Input: dimensioned drawing with shaded views. Units: mm. Origin: part minimum x, y, z. A direction names the side the tool comes from. Round coordinates to 2 decimals unless told otherwise and drop trailing zeros. Loops run counter-clockwise (first coordinate to the right, second up) from the corner with the lowest first, then second, coordinate; pieces in that order, holes last. Notation, with made-up numbers: (-3, 60.25) - (5, 60.25) arc R21 ccw to (5, 68.25) - close; hole circle Ø3 at (25.5, 39.25). An arc over 180 degrees is marked (long way). One line per question, with ' | ' between items.
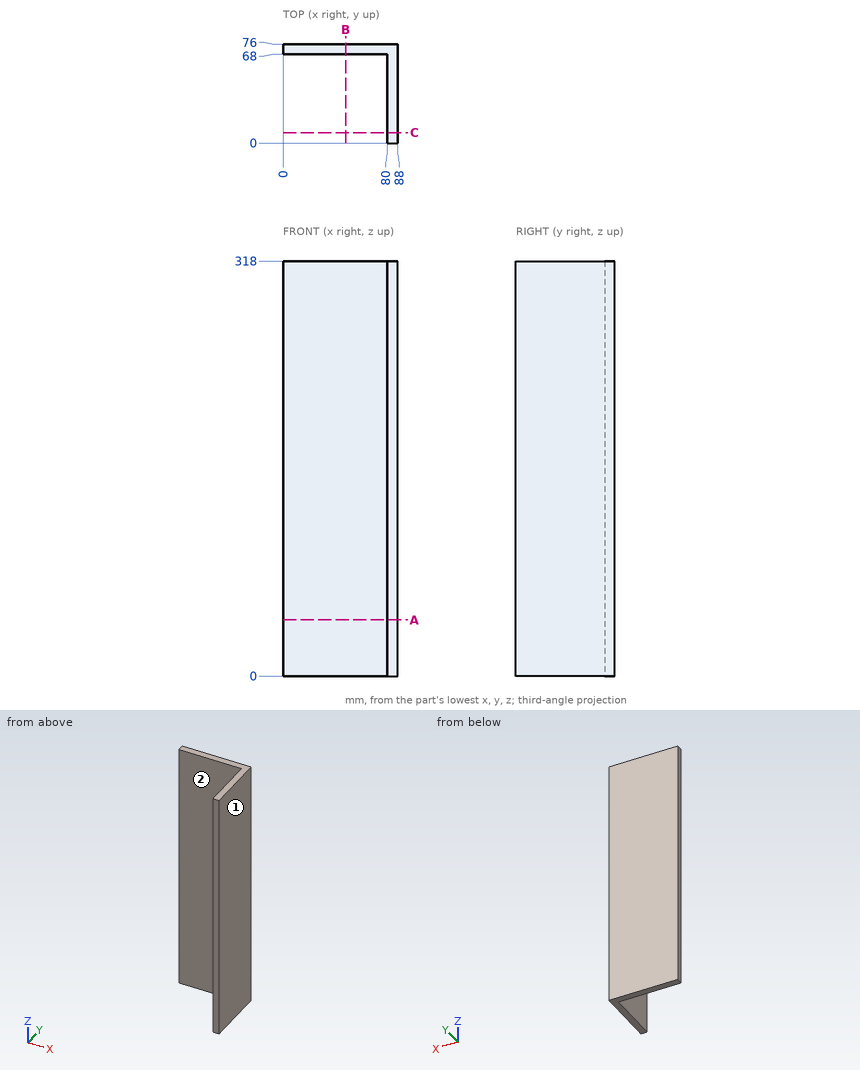
1. Contact query for a flat-ended pin moving along its axis: P1, Ø12, axis at y = 38.5, z = 45.5, coming from the -X side. Output: stop coordinate, or through.
Worked out:
P1: stops at x = 80
2. Section query B-B, the plane x = 48. Return loops of the section in (y, z), plus the area to 3 significant figures.
Worked out:
outline: (68, 0) - (76, 0) - (76, 318) - (68, 318) - close | area: 2,540 mm2
3. Access query for the marked faces 1 and 2. Directions: +Z, -Z, +X, -X, +Y, -Y. A direction counts if a zero-diameter tool reaches every point of the face in a straight line with its end or side. Return the directions, or none.
Worked out:
face 1: +Z, -Z, +X, +Y, -Y | face 2: +Z, -Z, -X, -Y
4. Section query C-C, the plane y = 8. Return loops of the section in (x, z).
Worked out:
outline: (80, 0) - (88, 0) - (88, 318) - (80, 318) - close
5. Material intervals for probe 1 along Y at (x, z) = (44, 27); probe 2 along X at (y, z) = (42, 231.5), sorted ascending.
Worked out:
probe 1: y = 68 to 76 | probe 2: x = 80 to 88
6. Section query A-A, the plane z = 43. Return loops of the section in (x, y).
Worked out:
outline: (0, 68) - (80, 68) - (80, 0) - (88, 0) - (88, 76) - (0, 76) - close
